For this review, take the finished solid that the model builds, in its own axes (mm). Face numbers are marked on the shaded views. A direction names the side the tool comes from. Coordinates: 2 decimals unless noted, no trailing zeros. Order: outer loops, then holes, each group sorted by start corner. A loop starts at its lowest first (then second) coordinate and runs counter-clockwise, first axis right, second up. Notation, with made-up numbers: (-30, -33.75) -> (-3, -33.75) arc R12 ccw to (-3, -11.75) -> close; hole circle Ø2 at (85, -25.75). An arc over 180 degrees is marked (long way). Return JSON: item names as keys, results as strings. Group by question number.
Item 1: Machinability: for the marked faces 1, 2 and 3, which of the approach directions +Z, -Z, +X, -X, +Y, -Y give a long, thin tool a straight path to every point of the face, cutting with its end or side? Answer none if there is none.
Item 2: Insertion check: pin 1 (3 mm diameter, centred on y = 3.5, z = 0.5, fed in from -X); pin 2 (3 mm diameter, centred on y = 1, z = -3, fed in from -X); pin 3 (1 mm diameter, centred on y = -1.5, z = 3.5, fed in from +X). Each pin has a flat end and moves straight along its axis. Give the tip position at first contact, or say it passes through.
Item 3: For line 1 along Y through (x, z) = (-1.5, -1.5); line 2 along Z through (x, y) = (-2, -2); line 3 along Z through (x, y) = (-1, 1.5), list the stretches that pass through material, from the lowest coordinate up.
Item 4: Draft analysis for pull direction X (two halves, no side actions). For the marked faces 4, 5 and 6, state which applies: +X half, -X half, draft (parallel to the pull), parting line (faces both ways), or undercut.
Item 5: Take a section at A-A (y = 0). Write out the cut boundary in (x, z), then the cut area to 3 significant figures.
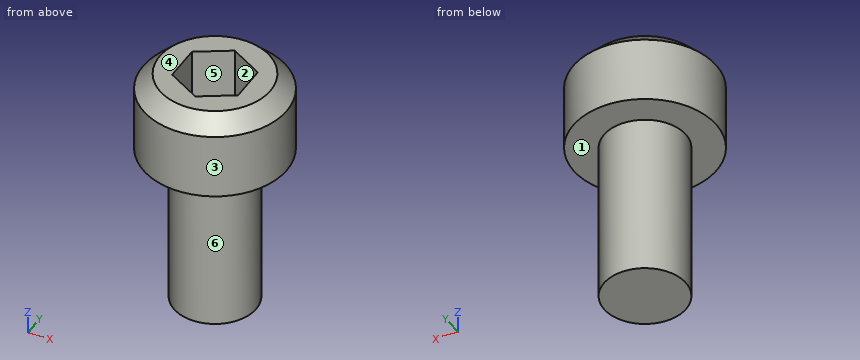
```python
from build123d import *

# Parameters (mm, degrees)
SKETCH_1_R          = 4.36
EXTRUDE_1_DEPTH     = 5
CUT_EXTRUDE_1_DEPTH = 4
CHAMFER_1_SIZE      = 1
SKETCH_3_R          = 2.5
EXTRUDE_2_DEPTH     = 10


with BuildPart() as part:
    # 草图1 → 凸台-拉伸1 (new body)
    with BuildSketch(Plane.XY):
        Circle(SKETCH_1_R)
    extrude(amount=EXTRUDE_1_DEPTH)

    # 草图2 → 切除-拉伸1 (cut)
    with BuildSketch(Plane.XY.offset(5)):
        Polygon((0, 2.309401077), (-2, 1.154700538), (-2, -1.154700538), (0, -2.309401077), (2, -1.154700538), (2, 1.154700538), align=None)
    extrude(amount=-CUT_EXTRUDE_1_DEPTH, mode=Mode.SUBTRACT)

    # 倒角1
    chamfer_1_edges = [part.edges().sort_by_distance(p)[0] for p in [
        (-4.36, 0, 5),
    ]]
    chamfer(chamfer_1_edges, length=CHAMFER_1_SIZE)

    # 草图3 → 凸台-拉伸2 (add)
    with BuildSketch(Plane(origin=(0, 0, 0), x_dir=(-1, 0, 0), z_dir=(0, 0, -1))):
        with Locations(Location((0, 0, 0), (0, 0, 180))):
            Circle(SKETCH_3_R)
    extrude(amount=EXTRUDE_2_DEPTH)


solid = part.part
```
Findings below:
{
 "1": {"face 1": "-Z", "face 2": "+Z", "face 3": "+Z, -Z"},
 "2": {"pin 1": "stops at x = -3.87", "pin 2": "stops at x = -2.5", "pin 3": "stops at x = 4.24"},
 "3": {"line 1": "y = -2 to 2", "line 2": "z = 0 to 5", "line 3": "z = -10 to 1"},
 "4": {"face 4": "draft", "face 5": "undercut", "face 6": "parting line"},
 "5": {"outline": "(-4.36, 0) -> (-2.5, 0) -> (-2.5, -10) -> (2.5, -10) -> (2.5, 0) -> (4.36, 0) -> (4.36, 4) -> (3.36, 5) -> (2, 5) -> (2, 1) -> (-2, 1) -> (-2, 5) -> (-3.36, 5) -> (-4.36, 4) -> close", "area": "76.6 mm2"}
}
